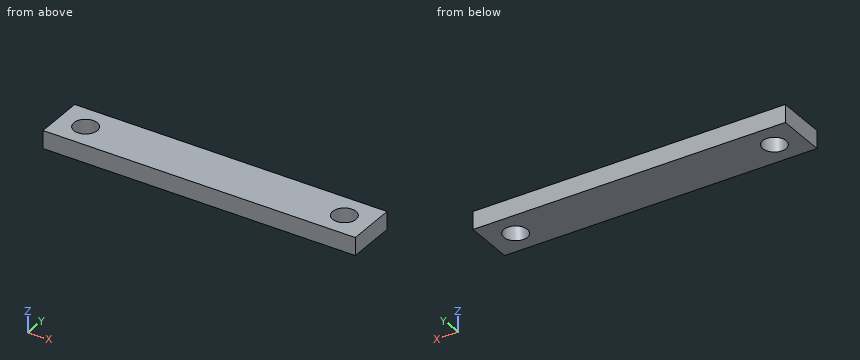
```python
from build123d import *

# Parameters (mm, degrees)
SKETCH1_W           = 140
SKETCH1_H           = 22
BOSS_EXTRUDE1_DEPTH = 8
SKETCH2_R           = 5.25
CUT_EXTRUDE1_DEPTH  = 79.751224998


with BuildPart() as part:
    # Sketch1 → Boss-Extrude1 (new body)
    with BuildSketch(Plane.XY):
        with Locations((0.089565278, 24.00297527)):
            Rectangle(SKETCH1_W, SKETCH1_H)
    extrude(amount=BOSS_EXTRUDE1_DEPTH)

    # Sketch2 → Cut-Extrude1 (cut, through all)
    with BuildSketch(Plane.XY.offset(8)):
        with Locations((-57.910434722, 24.00297527)):
            Circle(SKETCH2_R)
        with Locations(Location((58.089565278, 24.00297527, 0), (0, 0, 180))):
            Circle(SKETCH2_R)
    extrude(amount=-CUT_EXTRUDE1_DEPTH, mode=Mode.SUBTRACT)


solid = part.part
```
Could you check a few things on this model? Use its own coordinates, in mm. Give positions to 0.01 mm unless a question says otherwise; leave off trailing zeros. Write each loop counter-clockwise with the first axis right and the second up, starting at its lowest first coordinate (ties: lowest second). Pieces come first, ordered by that corner, then holes. Notation, with made-up numbers: (58.25, 30) - (74.25, 30) arc R8 ccw to (74.25, 45) - close; hole circle Ø5 at (-30, 55.5). An arc over 180 degrees is marked (long way). One line per item, written item: value. Start each with the question number.
Item 1: Imagine slicing it at B-B, the plane y = 27.5. List the corners of the cut face in (x, z) for me, and give its area (3 significant figures).
Item 2: Please list where these lines run through material, in increasing order: line 1 (X direction, y = 28.5, z = 1); line 2 (X direction, y = 21.5, z = 7.75); line 3 (Y direction, x = -57, z = 5.25). Write a range as from..to.
Item 3: Imagine slicing it at C-C, the plane z = 1.25. List the corners of the cut face in (x, y) for me.
Item 4: Imagine slicing it at A-A, the plane x = 56.5. List the corners of the cut face in (y, z) for me.
Item 5: I'm going to push a flat-ended pin straight in: pin 1 (9.5 mm diameter, centred on x = -57.91, y = 24, fed in from -Z). Where does the tip first touch, or does it pass through?
Geometry says:
1. outline: (-69.91, 0) - (-61.83, 0) - (-61.83, 8) - (-69.91, 8) - close; (-53.99, 0) - (54.17, 0) - (54.17, 8) - (-53.99, 8) - close; (62.01, 0) - (70.09, 0) - (70.09, 8) - (62.01, 8) - close
1. area: 995 mm^2
2. line 1: -69.91..-60.62, -55.2..55.38, 60.8..70.09
2. line 2: -69.91..-62.53, -53.3..53.47, 62.7..70.09
2. line 3: 13..18.83, 29.17..35
3. outline: (-69.91, 13) - (70.09, 13) - (70.09, 35) - (-69.91, 35) - close; hole circle Ø10.5 at (-57.91, 24); hole circle Ø10.5 at (58.09, 24)
4. outline: (13, 0) - (19, 0) - (19, 8) - (13, 8) - close; (29.01, 0) - (35, 0) - (35, 8) - (29.01, 8) - close
5. pin 1: through
